```python
from build123d import *

# Parameters (mm, degrees)
FLANGE_PLATE_DEPTH            = 7.5
HUB_SKETCH_R                  = 25
HUB_50_DEPTH                  = 55
HUB_BORE_SKETCH_R             = 15
HUB_BORE_30_DEPTH             = 120.353625921
SLOTTED_START                 = 15
SLOTTED_COLLAR_SKETCH_R       = 15
SLOTTED_COLLAR_DEPTH          = 15
GUSSET_DEPTH                  = 7.5
COLLAR_FACE_BOSS_SKETCH_R     = 15
COLLAR_FACE_BOSS_DEPTH        = 85
THROUGH_BORE_20_SKETCH_R      = 10
THROUGH_BORE_20_DEPTH         = 132.416467844
COLLAR_BORE_30_SKETCH_R       = 15
COLLAR_BORE_30_DEPTH_45_DEPTH = 45


with BuildPart() as part:
    # Flange Plate Sketch → Flange Plate (new, symmetric)
    with BuildSketch(Plane.XY):
        with BuildLine():
            Line((-80, 30), (80, 30))
            ThreePointArc((80, 30), (89.443039653, 20.328945287), (91.687925992, 7))
            Line((91.687925992, 7), (60, 7))
            ThreePointArc((60, 7), (53, 0), (60, -7))
            Line((60, -7), (91.687925992, -7))
            ThreePointArc((91.687925992, -7), (89.443039653, -20.328945287), (80, -30))
            Line((80, -30), (-80, -30))
            ThreePointArc((-80, -30), (-89.443039653, -20.328945287), (-91.687925992, -7))
            Line((-91.687925992, -7), (-60, -7))
            ThreePointArc((-60, -7), (-53, 0), (-60, 7))
            Line((-60, 7), (-91.687925992, 7))
            ThreePointArc((-91.687925992, 7), (-89.443039653, 20.328945287), (-80, 30))
        make_face()
    extrude(amount=FLANGE_PLATE_DEPTH, both=True)

    # Hub Sketch → Hub Ø50 (add)
    with BuildSketch(Plane.XY.offset(7.5)):
        with Locations(Location((0, 0, 0), (0, 0, 180))):
            Circle(HUB_SKETCH_R)
    extrude(amount=HUB_50_DEPTH)

    # Hub Bore Sketch → Hub Bore Ø30 (cut, through all)
    with BuildSketch(Plane.XY.offset(62.5)):
        Circle(HUB_BORE_SKETCH_R)
    extrude(amount=-HUB_BORE_30_DEPTH, mode=Mode.SUBTRACT)

    # Slotted Collar Sketch → Slotted Collar (add)
    with BuildSketch(Plane.XY.offset(62.5).offset(SLOTTED_START)):
        with BuildLine():
            ThreePointArc((3, -25), (4.414213562, -25.585786438), (5, -27))
            Line((5, -27), (5, -40))
            Line((5, -40), (10, -40))
            ThreePointArc((10, -40), (25.27864045, 0), (10, 40))
            Line((10, 40), (5, 40))
            Line((5, 40), (5, 27))
            ThreePointArc((5, 27), (4.414213562, 25.585786438), (3, 25))
            Line((3, 25), (-3, 25))
            ThreePointArc((-3, 25), (-4.414213562, 25.585786438), (-5, 27))
            Line((-5, 27), (-5, 40))
            Line((-5, 40), (-10, 40))
            ThreePointArc((-10, 40), (-25.27864045, 0), (-10, -40))
            Line((-10, -40), (-5, -40))
            Line((-5, -40), (-5, -27))
            ThreePointArc((-5, -27), (-4.414213562, -25.585786438), (-3, -25))
            Line((-3, -25), (3, -25))
        make_face()
        Circle(SLOTTED_COLLAR_SKETCH_R, mode=Mode.SUBTRACT)
    extrude(amount=-SLOTTED_COLLAR_DEPTH)

    # Gusset Sketch → Gusset (add, symmetric)
    with BuildSketch(Plane(origin=(0, 0, 0), x_dir=(1, 0, 0), z_dir=(0, 1, 0))):
        Polygon((-24.85288252, -7.5), (-24.85288252, -42.5), (-49.85288252, -7.5), align=None)
    gusset = extrude(amount=GUSSET_DEPTH, both=True)

    # Gusset Mirror: Gusset across plane
    add(gusset.mirror(Plane(origin=(0, 0, 0), x_dir=(0, 0, 1), z_dir=(1, 0, 0))))

    # Collar Face Boss Sketch → Collar Face Boss (add, through all)
    with BuildSketch(Plane.XY.offset(77.5)):
        Circle(COLLAR_FACE_BOSS_SKETCH_R)
    extrude(amount=-COLLAR_FACE_BOSS_DEPTH)

    # Through Bore Ø20 Sketch → Through Bore Ø20 (cut, through all)
    with BuildSketch(Plane.XY.offset(77.5)):
        Circle(THROUGH_BORE_20_SKETCH_R)
    extrude(amount=-THROUGH_BORE_20_DEPTH, mode=Mode.SUBTRACT)

    # Collar Bore Ø30 Sketch → Collar Bore Ø30 Depth 45 (cut)
    with BuildSketch(Plane.XY.offset(77.5)):
        Circle(COLLAR_BORE_30_SKETCH_R)
    extrude(amount=-COLLAR_BORE_30_DEPTH_45_DEPTH, mode=Mode.SUBTRACT)


solid = part.part
```
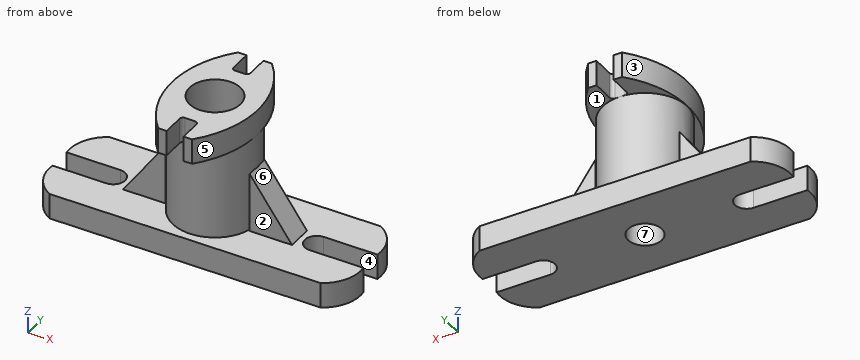
Geometry: final body of the model. Coordinates: model frame, mm. Face numbers are marked on the shaded views. A direction names the side the tool comes from. Coordinates: 2 decimals unless noted, no trailing zeros. Write each loop counter-clockwise with the first axis right and the second up, starting at its lowest first coordinate (ties: lowest second). Pieces come first, ordered by that corner, then holes. Notation, with made-up numbers: M 50,82.25 L 95,82.25 A14 cw 95,102.25 Z; hole C 58.25,-15 d1. An arc over 180 degrees is marked long. Answer as CSV lines item,"result". Start each with the question number.
Q1. Reachability of the marked faces 1, 2, 3 and 4 from +Z, -Z, +X, -X, +Y, -Y: full face, straight path, thin tool, end or side. Return the list, or none.
Q2. Cut plane D-D on y = -23. Return the cut outline in (x, z), then the cut area to 3 significant figures.
Q3. Pin query (flat end, axial travel): P1, Ø20, axis at x = -40, z = 27.5, coming from the +Y side; P2, Ø10, axis at y = -3, z = 59.5, coming from the +X side; P3, Ø1, axis at y = 5.5, z = 24.5, coming from the -X side; P4, Ø1.5, axis at x = 27.5, z = 67.5, coming from the +Y side. Return the tip coordinate at first contact, or that it passes through.
Q4. Line query: line 1 (Y direction, x = 0, z = 18.5); line 2 (Y direction, x = 0, z = 67); line 3 (Z direction, x = -71, y = -23). Output: solid intervals per line, ascending. Write a range as from..to.
Q5. Cut plane C-C on x = 23. Return the cut outline in (y, z), then the cut area to 3 significant figures.
Q6. Mould query, pull axis Y, two halves, no side actions, for the marked faces 5, 6 and 7. Classes: released by +Y, released by -Y, zero draft, split by the parting line, or undercut.
Q7. Cut plane B-B on z = 39. Return the cut outline in (x, y), then the cut area to 3 significant figures.
Q8. Cut plane A-A on y = 0. Return the cut outline in (x, z).
Findings below:
1,face 1,"+X"
1,face 2,"+Z, +X, -Y"
1,face 3,"+Z, -X"
1,face 4,"+Z, -Z, +X"
2,outline,"M -87.85,-7.5 L 87.85,-7.5 L 87.85,7.5 L 9.8,7.5 L 9.8,62.5 L 20.7,62.5 L 20.7,77.5 L -20.7,77.5 L -20.7,62.5 L -9.8,62.5 L -9.8,7.5 L -87.85,7.5 Z"
2,area,"4,330 mm2"
3,P1,"stops at y = 7.5"
3,P2,"stops at x = 25.28"
3,P3,"stops at x = -38.07"
3,P4,"passes through"
4,line 1,"y = -25..-10, 10..25"
4,line 2,"y = -25..-15, 15..25"
4,line 3,"z = -7.5..7.5"
5,outline,"M -30,-7.5 L 30,-7.5 L 30,7.5 L 9.8,7.5 L 9.8,62.5 L 16.38,62.5 L 16.38,77.5 L -16.38,77.5 L -16.38,62.5 L -9.8,62.5 L -9.8,7.5 L -30,7.5 Z"
5,area,"2,470 mm2"
6,face 5,"split by the parting line"
6,face 6,"zero draft"
6,face 7,"undercut"
7,outline,"M -27.35,-7.5 L -24.85,-7.5 L -24.85,-2.71 A25 ccw 24.85,-2.71 L 24.85,-7.5 L 27.35,-7.5 L 27.35,7.5 L 24.85,7.5 L 24.85,2.71 A25 ccw -24.85,2.71 L -24.85,7.5 L -27.35,7.5 Z; hole C 0,0 d30"
7,area,"1,330 mm2"
8,outline,"M -53,-7.5 L -10,-7.5 L -10,32.5 L -15,32.5 L -15,77.5 L -25.28,77.5 L -25.28,62.5 L -25,62.5 L -25,42.29 L -49.85,7.5 L -53,7.5 Z; M 10,-7.5 L 53,-7.5 L 53,7.5 L 49.85,7.5 L 25,42.29 L 25,62.5 L 25.28,62.5 L 25.28,77.5 L 15,77.5 L 15,32.5 L 10,32.5 Z"
